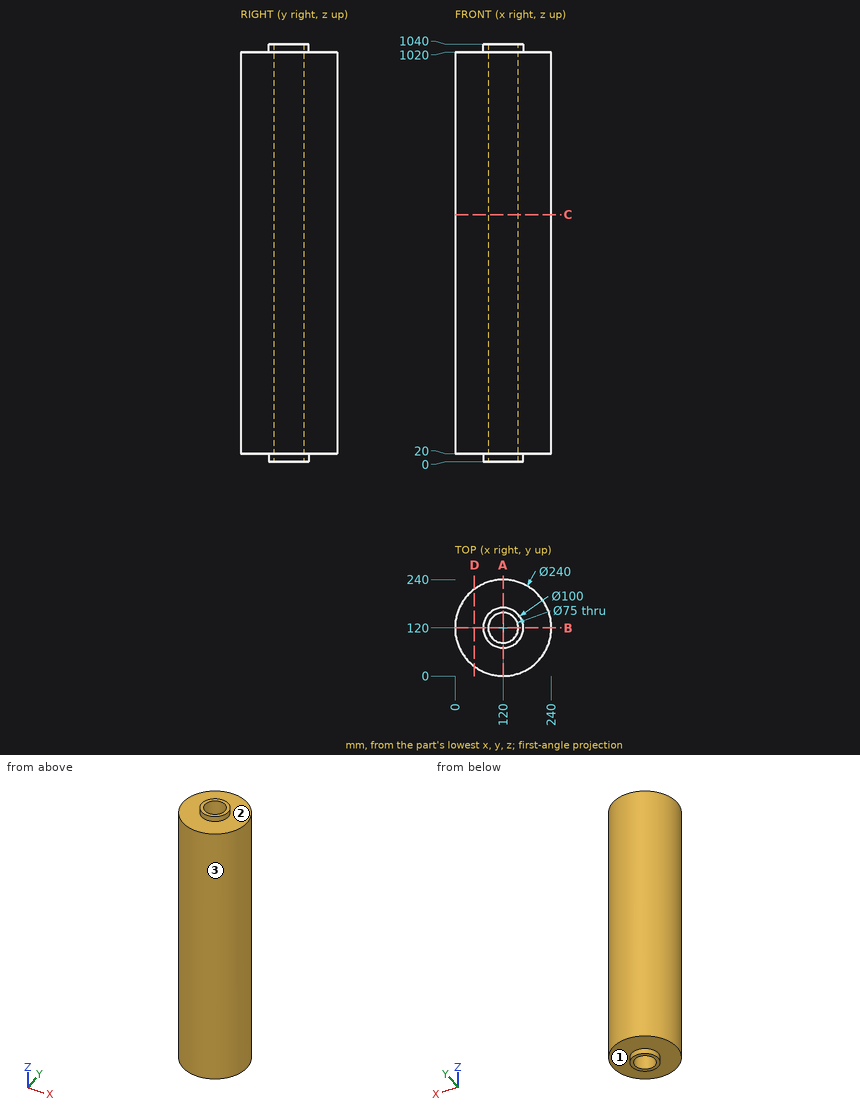
For this review, use the dimensioned drawing (mm, ordinates from the lowest corner) and the shaded views. A direction names the side the tool comes from. Give positions to 0.01 mm unless a question says otherwise; leave off trailing zeros. Loops run counter-clockwise (first coordinate to the right, second up) from the corner with the lowest first, then second, coordinate; pieces in that order, holes last.
Item 1: Take a section at D-D, the plane x = 48. State the section outline as (y, z) points, and give its area (3 significant figures).
Item 2: Tool access review of the marked faces 1, 2 and 3: name each direction out of +Z, -Z, +X, -X, +Y, -Y from which nothing blocks a thin tool from reaching the whole face with its end or side.
Item 3: Take a section at A-A, the plane x = 120. State the section outline as (y, z) points, and give its area (3 significant figures).
Item 4: For line 1 along Y through (x, z) = (120, 550); line 2 along Z through (x, y) = (213, 58); line 3 along Y through (x, z) = (126.5, 288), list the stretches that pass through material, from the lowest coordinate up.
Item 5: Take a section at C-C, the plane z = 615. State the section outline as (x, y) points, and give its area (3 significant figures).
Item 6: Insertion check: pin 1 (10 mm diameter, centred on y = 31.5, z = 607, fed in from -X); pin 2 (1.5 mm diameter, centred on y = 142.5, z = 180.5, fed in from +X); pin 3 (8 mm diameter, centred on x = 49.5, y = 168.5, fed in from -Z). Each pin has a flat end and moves straight along its axis. Give the tip position at first contact, or say it passes through.
Calculated:
1. outline: (24, 20) - (216, 20) - (216, 1020) - (24, 1020) - close
1. area: 192,000 mm2
2. face 1: -Z
2. face 2: +Z
2. face 3: +Z, -Z
3. outline: (0, 20) - (70, 20) - (70, 0) - (82.5, 0) - (82.5, 1040) - (70, 1040) - (70, 1020) - (0, 1020) - close; (157.5, 0) - (170, 0) - (170, 20) - (240, 20) - (240, 1020) - (170, 1020) - (170, 1040) - (157.5, 1040) - close
3. area: 166,000 mm2
4. line 1: y = 0 to 82.5, 157.5 to 240
4. line 2: z = 20 to 1020
4. line 3: y = 0.18 to 83.07, 156.93 to 239.82
5. outline: circle Ø240 at (120, 120); hole circle Ø75 at (120, 120)
5. area: 40,800 mm2
6. pin 1: stops at x = 33.82
6. pin 2: stops at x = 238.01
6. pin 3: stops at z = 20
